```python
from build123d import *

# Parameters (mm, degrees)
SKETCH_1_R        = 1
EXTRUDE_952_DEPTH = 1.2


with BuildPart() as part:
    # 草图1 → Extrude 952 (new body)
    with BuildSketch(Plane.XY):
        with BuildLine():
            Line((-6.468002299, -6.001541065), (-3.669934116, -8.860004717))
            Line((-3.669934116, -8.860004717), (-5.338433881, -12.888119479))
            ThreePointArc((-5.338433881, -12.888119479), (0, 13.95), (5.338433881, -12.888119479))
            Line((5.338433881, -12.888119479), (3.669934116, -8.860004717))
            Line((3.669934116, -8.860004717), (6.468002299, -6.001541065))
            ThreePointArc((6.468002299, -6.001541065), (9.014108926, -6.738296556), (11.033790366, -5.021801727))
            ThreePointArc((11.033790366, -5.021801727), (0, 11.15), (-11.033790366, -5.021801727))
            ThreePointArc((-11.033790366, -5.021801727), (-9.014108926, -6.738296556), (-6.468002299, -6.001541065))
        make_face()
        with Locations((-6.298089329, -9.978680815)):
            Circle(SKETCH_1_R, mode=Mode.SUBTRACT)
        with Locations(Location((6.298089329, -9.978680815, 0), (0, 0, 180))):
            Circle(SKETCH_1_R, mode=Mode.SUBTRACT)
    extrude(amount=EXTRUDE_952_DEPTH)


solid = part.part
```
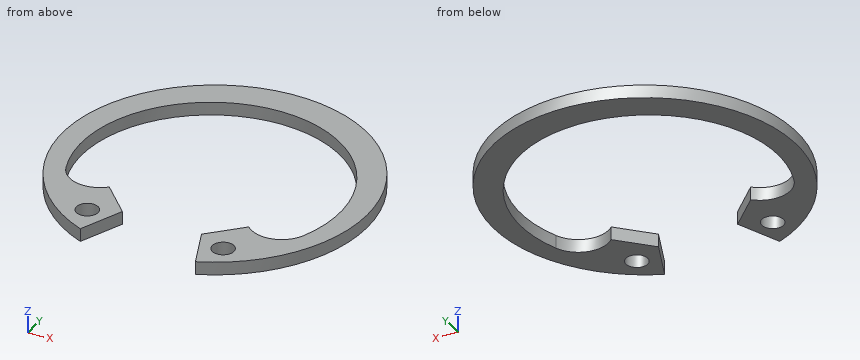
For this review, take the finished solid that the model builds, in its own axes (mm). Round coordinates to 2 decimals unless told otherwise and drop trailing zeros. Write each loop counter-clockwise with the first axis right and the second up, starting at its lowest first coordinate (ties: lowest second). Pieces come first, ordered by that corner, then holes. Notation, with made-up numbers: (77.5, -22) - (114.5, -22) arc R24 cw to (114.5, -2) - close; hole circle Ø2 at (74.25, -3.75). An arc over 180 degrees is marked (long way). Answer as CSV lines item,"result". Start each with the question number.
(1) Add section D-D, the plane x = 0. State the section outline as (y, z) points.
(2) Add section A-A, the plane y = -8.5. State the section outline as (x, z) points.
(3) For pin 1 (1.8 mm diameter, centred on x = -6.3, y = -9.98, fed in from -Z); pin 2 (12 mm diameter, centred on x = 11, y = -3.5, fed in from -Z), all flat-tipped, find the tip position at first contact; note any pin that passes through.
(4) For line 1 (Y direction, x = 7, z = 0.2); line 2 (Y direction, x = 6, z = 0.35); line 3 (Y direction, x = -0.25, z = 1.1), list the stretches that pass through material, from the lowest coordinate up.
(5) Add section C-C, the plane y = 9.5. State the section outline as (x, z) points, plus the area to 3 significant figures.
(6) Add section B-B, the plane z = 0.9. State the section outline as (x, y) points, plus the area to 3 significant figures.
From the geometry:
1,outline,"(11.15, 0) - (13.95, 0) - (13.95, 1.2) - (11.15, 1.2) - close"
2,outline,"(-11.06, 0) - (-4.02, 0) - (-4.02, 1.2) - (-11.06, 1.2) - close; (4.02, 0) - (11.06, 0) - (11.06, 1.2) - (4.02, 1.2) - close"
3,pin 1,"passes through"
3,pin 2,"stops at z = 0"
4,line 1,"y = -12.07 to -10.69, -9.27 to -6.41, 8.86 to 12.07"
4,line 2,"y = -12.59 to -10.93, -9.02 to -6.48, 9.52 to 12.59"
4,line 3,"y = 11.15 to 13.95"
5,outline,"(-10.22, 0) - (-6.03, 0) - (-6.03, 1.2) - (-10.22, 1.2) - close; (6.03, 0) - (10.22, 0) - (10.22, 1.2) - (6.03, 1.2) - close"
5,area,"10.0 mm²"
6,outline,"(-11.03, -5.02) arc R11.85 cw (long way) to (11.03, -5.02) arc R2.8 cw to (6.47, -6) - (3.67, -8.86) - (5.34, -12.89) arc R13.95 ccw (long way) to (-5.34, -12.89) - (-3.67, -8.86) - (-6.47, -6) arc R2.8 cw to start; hole circle Ø2 at (-6.3, -9.98); hole circle Ø2 at (6.3, -9.98)"
6,area,"186 mm²"
